```python
from build123d import *

# Parameters (mm, degrees)
G1_1_4_TAPPED_HOLE1_D     = 39.25
G1_1_4_TAPPED_HOLE1_DEPTH = 90.75
G1_1_4_TAPPED_HOLE1_TIP   = 11.791889648
CHAMFER1_SIZE             = 2


with BuildPart() as part:
    # Sketch1 → Revolve1 (revolve)
    with BuildSketch(Plane.XY, mode=Mode.PRIVATE) as revolve1_sk:
        Polygon((0, 0), (30, 0), (30, -12), (25, -12), (25, -20), (0, -20), align=None)
    revolve(revolve1_sk.sketch.rotate(Axis((0, -20, 0), (0, 1, 0)), 90), axis=Axis((0, -20, 0), (0, 1, 0)))

    # G1-1/4 Tapped Hole1
    with Locations(Plane(origin=(0, 0, 0), x_dir=(1, 0, 0), z_dir=(0, 1, 0))):
        with Locations((0, 0)):
            Hole(G1_1_4_TAPPED_HOLE1_D / 2, depth=G1_1_4_TAPPED_HOLE1_DEPTH)
            with Locations((0, 0, -(G1_1_4_TAPPED_HOLE1_DEPTH + G1_1_4_TAPPED_HOLE1_TIP / 2))):  # 118° drill point
                Cone(0, G1_1_4_TAPPED_HOLE1_D / 2, G1_1_4_TAPPED_HOLE1_TIP, mode=Mode.SUBTRACT)

    # Chamfer1
    chamfer1_edges = [part.edges().sort_by_distance(p)[0] for p in [
        (0, 0, 30),
    ]]
    chamfer(chamfer1_edges, length=CHAMFER1_SIZE)


solid = part.part
```
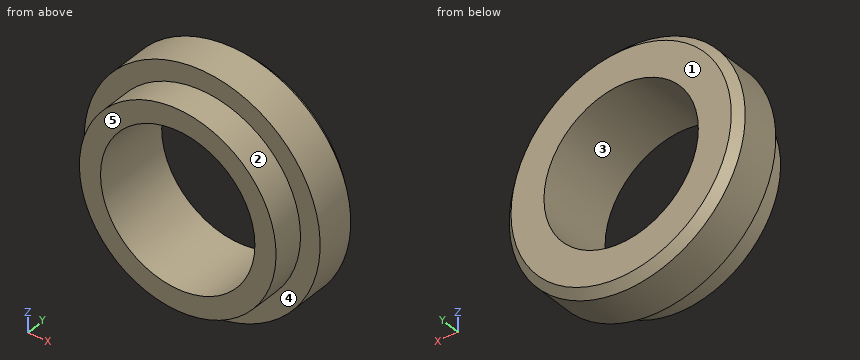
Read the model definition and answer for the solid it produces. Units are mm, in the model's axes. Face numbers are marked on the shaded views. A direction names the side the tool comes from. Round coordinates to 2 decimals unless told otherwise and drop trailing zeros. Write each loop counter-clockwise with the first axis right and the second up, starting at its lowest first coordinate (ties: lowest second). Pieces come first, ordered by that corner, then holes. Notation, with made-up numbers: (78, 31.5) -> (87, 31.5) arc R36 cw to (87, 68.5) -> close; hole circle Ø1 at (89.25, 88). An arc over 180 degrees is marked (long way). Answer in a Markdown table with one row per item. Add a question column.
1) Given P1, Ø4, axis at x = -1, y = -15.5, coming from the +Z side; P2, Ø4, axis at x = 3, y = -15, coming from the -Z side; P3, Ø3, axis at y = -4.5, z = 0.5, coming from the -X side, each flat-ended and moving along its own axis, determine where each tip first touches the part or whether it passes through.
2) Determine the mould class of the marked faces 1, 2 and 3 for opening direction X: pulls with the +X half, pulls with the -X half, needs draft (parallel to the pull), parting line crosses it, or undercut.
3) Find section C-C, the plane y = -12.75. Determine the outline of the cut face in (x, z) (3 decimals).
4) Which of the six approach directions +Z, -Z, +X, -X, +Y, -Y give full straight-line access (tool end or side, diameter ignored) to the marked faces 4 and 5?
5) Find section B-B, the plane x = 0. Determine the outline of the cut face in (y, z) (3 decimals).
6) Consider line 1 (Y direction, x = 20, z = 18); line 2 (X direction, y = -18.25, z = 17.5); line 3 (Z direction, x = 6, y = -4). Determine where each line is inside the solid, lowest interval first.
7) Find section A-A, the plane z = 0. Determine the outline of the cut face in (x, y) (3 decimals).
8) Find section D-D, the plane y = -4.5. Determine the outline of the cut face in (x, z) (3 decimals).
Findings below:
| question | item | result |
|---|---|---|
| 1 | P1 | z = 25 |
| 1 | P2 | z = -24.98 |
| 1 | P3 | x = -30 |
| 2 | face 1 | needs draft |
| 2 | face 2 | parting line crosses it |
| 2 | face 3 | undercut |
| 3 | outline | circle Ø50 at (0, 0); hole circle Ø39.25 at (0, 0) |
| 4 | face 4 | -Y |
| 4 | face 5 | +Z, -Z, +X, -X, -Y |
| 5 | outline | (-20, -25) -> (-12, -25) -> (-12, -30) -> (-2, -30) -> (0, -28) -> (0, -19.625) -> (-20, -19.625) -> close; (-20, 19.625) -> (0, 19.625) -> (0, 28) -> (-2, 30) -> (-12, 30) -> (-12, 25) -> (-20, 25) -> close |
| 6 | line 1 | -12 to 0 |
| 6 | line 2 | -17.85 to -8.88, 8.88 to 17.85 |
| 6 | line 3 | -29.39 to -18.69, 18.69 to 29.39 |
| 7 | outline | (-30, -12) -> (-25, -12) -> (-25, -20) -> (-19.625, -20) -> (-19.625, 0) -> (-28, 0) -> (-30, -2) -> close; (19.625, -20) -> (25, -20) -> (25, -12) -> (30, -12) -> (30, -2) -> (28, 0) -> (19.625, 0) -> close |
| 8 | outline | circle Ø60 at (0, 0); hole circle Ø39.25 at (0, 0) |
